```python
from build123d import *

# Parameters (mm, degrees)
MEMBER_1_DEPTH     = 598
HOLE_WIZARD_M5_1_D = 4.2


with BuildPart() as part:
    # Sketch1 → Member 1 (new body)
    with BuildSketch(Plane(origin=(0, 0, 0), x_dir=(0, 0, -1), z_dir=(1, 0, 0))):
        with BuildLine():
            Line((-9.8, -15), (9.8, -15))
            ThreePointArc((9.8, -15), (13.476955262, -13.476955262), (15, -9.8))
            Line((15, -9.8), (15, 9.8))
            ThreePointArc((15, 9.8), (13.476955262, 13.476955262), (9.8, 15))
            Line((9.8, 15), (-9.8, 15))
            ThreePointArc((-9.8, 15), (-13.476955262, 13.476955262), (-15, 9.8))
            Line((-15, 9.8), (-15, -9.8))
            ThreePointArc((-15, -9.8), (-13.476955262, -13.476955262), (-9.8, -15))
        make_face()
        with BuildLine():
            Line((-9.8, -12.4), (9.8, -12.4))
            ThreePointArc((9.8, -12.4), (11.638477631, -11.638477631), (12.4, -9.8))
            Line((12.4, -9.8), (12.4, 9.8))
            ThreePointArc((12.4, 9.8), (11.638477631, 11.638477631), (9.8, 12.4))
            Line((9.8, 12.4), (-9.8, 12.4))
            ThreePointArc((-9.8, 12.4), (-11.638477631, 11.638477631), (-12.4, 9.8))
            Line((-12.4, 9.8), (-12.4, -9.8))
            ThreePointArc((-12.4, -9.8), (-11.638477631, -11.638477631), (-9.8, -12.4))
        make_face(mode=Mode.SUBTRACT)
    extrude(amount=MEMBER_1_DEPTH)

    # M5 螺纹孔1 (through all)
    with Locations(Plane.XY.offset(15)):
        with Locations((355.000000009, 0), (245.000000009, 0)):
            Hole(HOLE_WIZARD_M5_1_D / 2)


solid = part.part
```
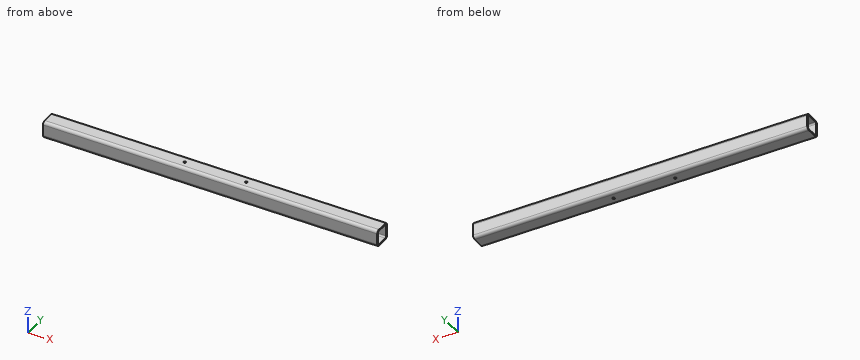
Geometry check sheet. Reference: the model listing, model coordinates, mm. Coordinates: 2 decimals unless noted, no trailing zeros. Loops run counter-clockwise (first coordinate to the right, second up) from the corner with the lowest first, then second, coordinate; pieces in that order, holes last. Notation, with made-up numbers: (68.5, 10) -> (110.5, 10) arc R30 cw to (110.5, 43) -> close; hole circle Ø5 at (33, 25.25). An arc over 180 degrees is marked (long way). Put each result on its own line as item: value.
1) Gauge pin test, flat end, axial feed: pin 1 Ø5 at (x, y) = (355, 0) entering from -Z. Record the tip position at first contact, or that the pin passes through.
Result set:
pin 1: stops at z = -15
2) Cross-section at B-B on z = -4.5. Record the boundary of the cut face in (x, y).
Result set:
outline: (0, -15) -> (598, -15) -> (598, -12.4) -> (0, -12.4) -> close; (0, 12.4) -> (598, 12.4) -> (598, 15) -> (0, 15) -> close
3) Cross-section at A-A on x = 255. Record the boundary of the cut face in (y, z).
Result set:
outline: (-15, -9.8) arc R5.2 ccw to (-9.8, -15) -> (9.8, -15) arc R5.2 ccw to (15, -9.8) -> (15, 9.8) arc R5.2 ccw to (9.8, 15) -> (-9.8, 15) arc R5.2 ccw to (-15, 9.8) -> close; hole (-12.4, -9.8) arc R2.6 ccw to (-9.8, -12.4) -> (9.8, -12.4) arc R2.6 ccw to (12.4, -9.8) -> (12.4, 9.8) arc R2.6 ccw to (9.8, 12.4) -> (-9.8, 12.4) arc R2.6 ccw to (-12.4, 9.8) -> close
4) Thickness scan on line 1 (Z direction, x = 348, y = -8.25); line 2 (Y direction, x = 355, z = 14.1). Record the ranges inside material, lowest first.
Result set:
line 1: z = -15 to -12.4, 12.4 to 15
line 2: y = -12.72 to -2.1, 2.1 to 12.72
